```python
from build123d import *

# Parameters (mm, degrees)
BASE_PLATE_DEPTH       = 5
RAISED_PAD_DEPTH       = 10
UPRIGHT_WALL_PROFILE_W = 10
UPRIGHT_WALL_PROFILE_H = 38
UPRIGHT_WALL_DEPTH     = 54
GUSSET_CUT_DEPTH       = 10


with BuildPart() as part:
    # Base Plate Profile → Base Plate (new, symmetric)
    with BuildSketch(Plane(origin=(0, 0, 0), x_dir=(1, 0, 0), z_dir=(0, 1, 0))):
        Polygon((0, 0), (81, 0), (125, 25), (125, 53), (0, 53), align=None)
    extrude(amount=BASE_PLATE_DEPTH, both=True)

    # Raised Pad Profile → Raised Pad (add)
    with BuildSketch(Plane(origin=(0, 0, -53), x_dir=(-1, 0, 0), z_dir=(0, 0, -1))):
        Polygon((-125, 5), (-10, 5), (-57, 59), (-125, 59), align=None)
    extrude(amount=-RAISED_PAD_DEPTH)

    # Upright Wall Profile → Upright Wall (add)
    with BuildSketch(Plane(origin=(0, 5, 0), x_dir=(1, 0, 0), z_dir=(0, 1, 0))):
        with Locations((75, 24)):
            Rectangle(UPRIGHT_WALL_PROFILE_W, UPRIGHT_WALL_PROFILE_H)
    extrude(amount=UPRIGHT_WALL_DEPTH)

    # Gusset Cut Profile → Gusset Cut (cut)
    with BuildSketch(Plane(origin=(80, 0, 0), x_dir=(0, 0, -1), z_dir=(1, 0, 0))):
        Polygon((43, 59), (5, 5), (5, 59), align=None)
    extrude(amount=-GUSSET_CUT_DEPTH, mode=Mode.SUBTRACT)


solid = part.part
```
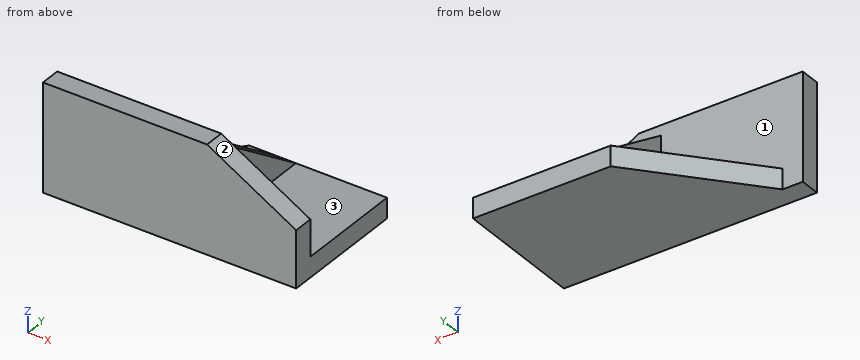
Work out the finished part from the listing and answer in its coordinate system (mm). Face numbers are marked on the shaded views. A direction names the side the tool comes from. Give positions to 0.01 mm unless a question says otherwise; leave off trailing zeros. Loops run counter-clockwise (first coordinate to the right, second up) from the corner with the lowest first, then second, coordinate; pieces in that order, holes last. Notation, with made-up numbers: (58.25, -17.75) -> (103.25, -17.75) arc R13 cw to (103.25, 7.25) -> close; hole circle Ø9 at (88, -18.5). An arc over 180 degrees is marked (long way). Use CSV: the item, a comma, the result in double quotes.
1. A tool of negligible diameter and unlimited length cuts with its end or side. For the marked faces 1, 2 and 3, from which of +Z, -Z, +X, -X, +Y, -Y can it reach the whole face along a straight path? Write none if from no direction.
Found:
face 1,"+Z, +Y"
face 2,"+Z, +X, +Y, -Y"
face 3,"+Z, +X, +Y"
2. The part is cut by section B-B (y = 19.5). Write down the section's boundary in (x, z).
Found:
outline,"(22.62, -53) -> (125, -53) -> (125, -43) -> (80, -43) -> (80, -15.2) -> (70, -15.2) -> (70, -43) -> (22.62, -43) -> close"
3. Straight lines are drawn through the part: line 1 (Y direction, x = 11, z = -31); line 2 (Z direction, x = 88.5, y = 15); line 3 (X direction, y = 19.5, z = -23). For each, find the intervals that lie inside material, in ascending order.
Found:
line 1,"-5 to 5"
line 2,"-53 to -43"
line 3,"70 to 80"
4. Flat-ended cylindrical pins translate along their axes: pin 1 Ø16 at (x, y) = (50.5, 27.5) entering from +Z; pin 2 Ø19 at (y, z) = (25.5, -19) entering from -X; pin 3 Ø6 at (x, z) = (66.5, -24) entering from +Y; pin 4 Ø2 at (x, y) = (25, 22.5) entering from -Z. Find the tip coordinate at first contact, or state that the pin passes through.
Found:
pin 1,"z = -43"
pin 2,"x = 70"
pin 3,"y = 5"
pin 4,"z = -53"
5. The part is cut by section C-C (x = 65). Write down the section's boundary in (y, z), then the cut area to 3 significant figures.
Found:
outline,"(-5, -53) -> (59, -53) -> (59, -43) -> (5, -43) -> (5, 0) -> (-5, 0) -> close"
area,"1,070 mm^2"
6. The part is cut by section D-D (z = -48). Write down the section's boundary in (x, y).
Found:
outline,"(0, -5) -> (125, -5) -> (125, 59) -> (57, 59) -> (10, 5) -> (0, 5) -> close"
7. The part is cut by section A-A (z = -33.5). Write down the section's boundary in (x, y).
Found:
outline,"(0, -5) -> (125, -5) -> (125, 5) -> (80, 5) -> (80, 45.5) -> (70, 45.5) -> (70, 5) -> (0, 5) -> close"
